Could you check a few things on this drawing? It's one solid part, dimensions in mm from its lowest x, y, z. Give positions to 0.01 mm unless a question says otherwise; leave off trailing zeros. Loops run counter-clockwise (first coordinate to the right, second up) from the corner with the lowest first, then second, coordinate; pieces in that order, holes last. Notation, with made-up numbers: (72.25, -33.75) - (130.25, -33.75) arc R27 cw to (130.25, 4.25) - close; hole circle Ø11 at (80.25, 60.25). An arc over 180 degrees is marked (long way). Return JSON: item names as keys, results as strings. Group by question number.
(1) If we mould it in two halves opening along X, with no side actions, what happens to the marked faces 1, 2, 3 and 4? For each: released by +X, released by -X, zero draft, split by the parting line, or undercut.
(2) I need wall thicknesses on probe 1 along X at (y, z) = (2.5, 35); probe 2 along X at (y, z) = (2.25, 33); probe 3 along Z at (x, y) = (91, 2.25). Which ranges of each line are inside material? Lowest first, please. Write a range as [from, to].
(3) If we section it at C-C (z = 35): Please give me the cut outline in (x, y).
(4) If we section it at B-B (y = 7): Please give me the cut outline in (x, z).
(5) If we section it at A-A (x = 20): Please give me the cut outline in (y, z), then the cut area to 3 significant figures.
(6) For P1, Ø12, axis at x = 46.5, z = 45.5, coming from the -Y side, with a flat end and sliding along its axis, tell me the tip position at first contact or that it passes through.
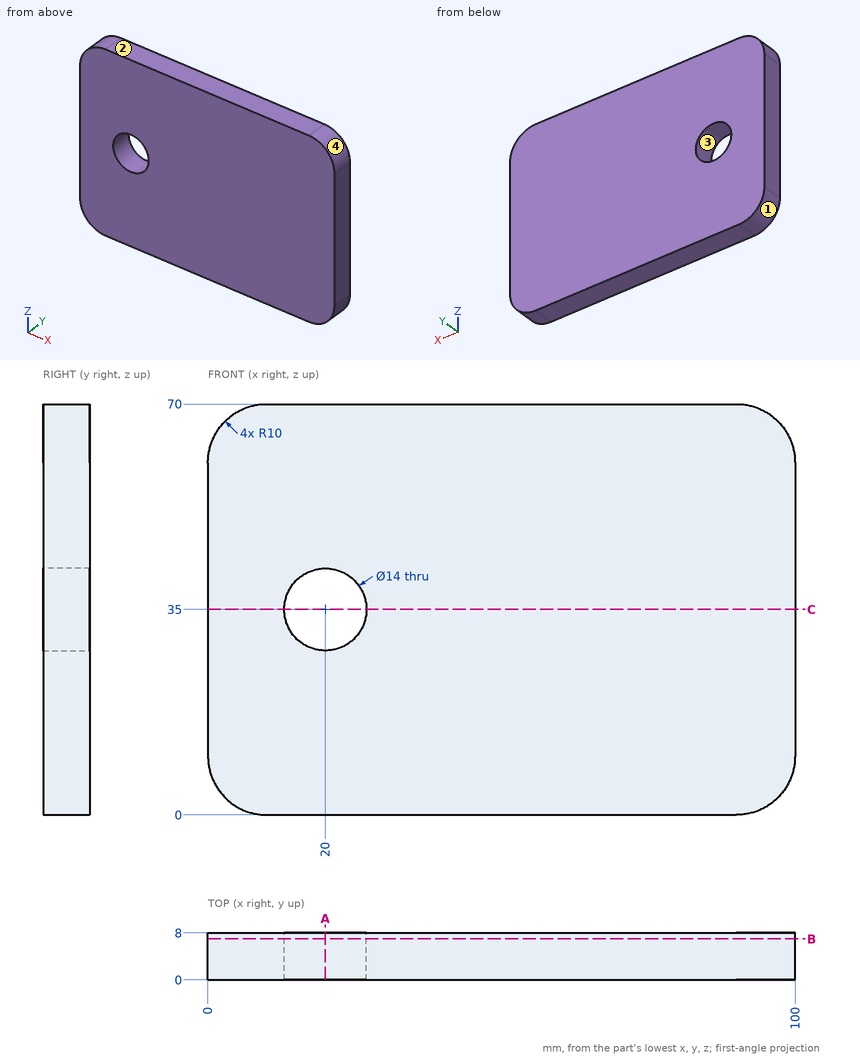
Values:
{
 "1": {"face 1": "released by -X", "face 2": "zero draft", "face 3": "undercut", "face 4": "released by +X"},
 "2": {"probe 1": "[0, 13], [27, 100]", "probe 2": "[0, 13.29], [26.71, 100]", "probe 3": "[0.05, 69.95]"},
 "3": {"outline": "(0, 0) - (13, 0) - (13, 8) - (0, 8) - close; (27, 0) - (100, 0) - (100, 8) - (27, 8) - close"},
 "4": {"outline": "(0, 10) arc R10 ccw to (10, 0) - (90, 0) arc R10 ccw to (100, 10) - (100, 60) arc R10 ccw to (90, 70) - (10, 70) arc R10 ccw to (0, 60) - close; hole circle Ø14 at (20, 35)"},
 "5": {"outline": "(0, 0) - (8, 0) - (8, 28) - (0, 28) - close; (0, 42) - (8, 42) - (8, 70) - (0, 70) - close", "area": "448 mm2"},
 "6": {"P1": "y = 0"}
}
